Job drawing, mm, ordinate dimensions from the low corner. One solid piece. A direction names the side the tool comes from. Give positions to 0.01 mm unless a question says otherwise; leave off trailing zeros. Write each loop counter-clockwise with the first axis right and the second up, starting at its lowest first coordinate (ties: lowest second). Pieces come first, ordered by that corner, then holes. Notation, with made-up numbers: M 1,63 L 21,63 A16 cw 21,67 Z; hole C 10,-19.75 d8. An arc over 180 degrees is marked long. Use CSV: the item, a comma, the result in double quotes. Start each with the question number.
Item 1: Mould opens along X. For the marked faces 1, 2 and 3 say: released by +X, released by -X, zero draft, split by the parting line, or undercut.
Item 2: Which spindle directions (+Z, -Z, +X, -X, +Y, -Y) get a long thin tool onto all of the face, cutting with end or side? Do the marked faces 4, 5 and 6. Say none if no direction does.
Item 3: Cut at B-B (z = 21). List the corners of the cut face in (x, y), then the cut area to 3 significant figures.
Item 4: Cut at D-D (y = 9). List the corners of the cut face in (x, z).
Item 5: Cut at A-A (y = 19). List the corners of the cut face in (x, z), then the cut area to 3 significant figures.
Item 6: Pin check, flat tips, straight feed: pin 1 (1.4 mm diameter, centred on x = 22.5, z = 16, fed in from -Y); pin 2 (3 mm diameter, centred on x = 14.5, z = 5.5, fed in from +Y); pin 3 (4 mm diameter, centred on x = 27.5, y = 22, fed in from +Z); pin 4 (1.5 mm diameter, centred on y = 18.5, z = 13, fed in from -X). Stop position of each tip, or through.
Item 7: Drill centre lines: line 1 (Z direction, x = 19.5, y = 9); line 2 (Y direction, x = 11, z = 2.5); line 3 (Y direction, x = 14.5, z = 8.75). Where is each one in solid material? Low to high. Write a range as [from, to].
Item 8: Cut at C-C (x = 19). List the corners of the cut face in (y, z), then the cut area to 3 significant figures.
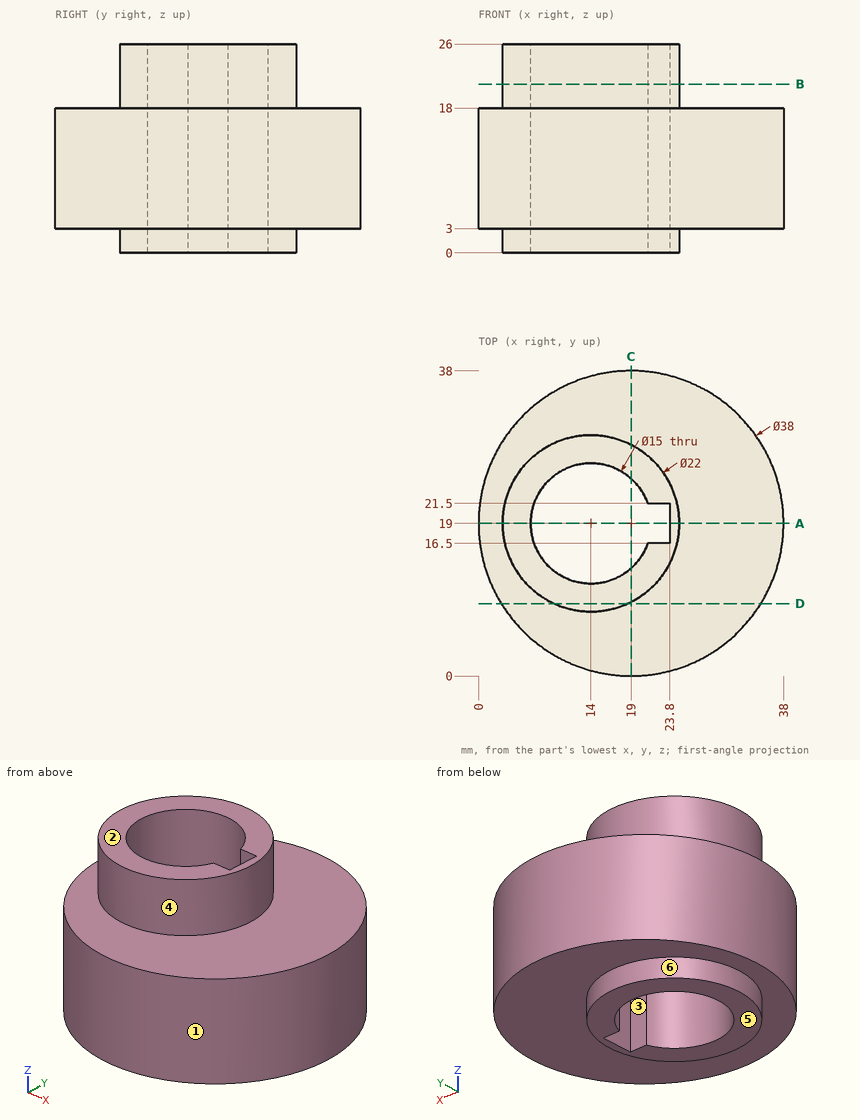
Worked answers:
1,face 1,"split by the parting line"
1,face 2,"zero draft"
1,face 3,"undercut"
2,face 4,"+Z"
2,face 5,"-Z, +X, -X, +Y, -Y"
2,face 6,"-Z"
3,outline,"C 14,19 d22; hole M 21.07,16.5 L 23.8,16.5 L 23.8,21.5 L 21.07,21.5 A7.5 ccw long Z"
3,area,"191 mm^2"
4,outline,"M 2.84,3 L 9.42,3 L 9.42,0 L 18.58,0 L 18.58,3 L 35.16,3 L 35.16,18 L 18.58,18 L 18.58,26 L 9.42,26 L 9.42,18 L 2.84,18 Z"
5,outline,"M 0,3 L 3,3 L 3,0 L 6.5,0 L 6.5,26 L 3,26 L 3,18 L 0,18 Z; M 23.8,0 L 25,0 L 25,3 L 38,3 L 38,18 L 25,18 L 25,26 L 23.8,26 Z"
5,area,"362 mm^2"
6,pin 1,"stops at y = 0.21"
6,pin 2,"stops at y = 37.76"
6,pin 3,"stops at z = 18"
6,pin 4,"stops at x = 0"
7,line 1,"z = [3, 18]"
7,line 2,"y = [8.42, 12.13], [25.87, 29.58]"
7,line 3,"y = [0.54, 11.52], [26.48, 37.46]"
8,outline,"M 0,3 L 9.2,3 L 9.2,0 L 13.41,0 L 13.41,26 L 9.2,26 L 9.2,18 L 0,18 Z; M 24.59,0 L 28.8,0 L 28.8,3 L 38,3 L 38,18 L 28.8,18 L 28.8,26 L 24.59,26 Z"
8,area,"495 mm^2"
